```python
from build123d import *

# Parameters (mm, degrees)
SKETCH_1_R      = 11.5
SKETCH_1_R_2    = 6.5
EXTRUDE_1_DEPTH = 14
SKETCH_2_R      = 19
SKETCH_2_R_2    = 6.5
EXTRUDE_2_DEPTH = 12
SKETCH_3_R      = 3.3
EXTRUDE_3_DEPTH = 4


with BuildPart() as part:
    # 草图1 → 拉伸1 (new body)
    with BuildSketch(Plane(origin=(0, 0, 0), x_dir=(1, 0, 0), z_dir=(0, 1, 0))):
        with Locations(Location((0, 0, 0), (0, 0, 270))):
            Circle(SKETCH_1_R)
        with Locations(Location((0, 0, 0), (0, 0, 270))):
            Circle(SKETCH_1_R_2, mode=Mode.SUBTRACT)
    extrude(amount=EXTRUDE_1_DEPTH)

    # 草图2 → 拉伸2 (add)
    with BuildSketch(Plane(origin=(0, 14, 0), x_dir=(-1, 0, 0), z_dir=(0, 1, 0))):
        with Locations(Location((0, 0, 0), (0, 0, 90))):
            Circle(SKETCH_2_R)
        with Locations(Location((0, 0, 0), (0, 0, 90))):
            Circle(SKETCH_2_R_2, mode=Mode.SUBTRACT)
    extrude(amount=EXTRUDE_2_DEPTH)

    # 草图3 → 拉伸3 (add)
    with BuildSketch(Plane(origin=(0, 26, 0), x_dir=(-1, 0, 0), z_dir=(0, 1, 0))):
        with Locations(Location((-15, 0, 0), (0, 0, 90))):
            Circle(SKETCH_3_R)
        with Locations(Location((0, -15, 0), (0, 0, 90))):
            Circle(SKETCH_3_R)
        with Locations(Location((0, 15, 0), (0, 0, 90))):
            Circle(SKETCH_3_R)
        with Locations(Location((15, 0, 0), (0, 0, 90))):
            Circle(SKETCH_3_R)
    extrude(amount=EXTRUDE_3_DEPTH)


solid = part.part
```
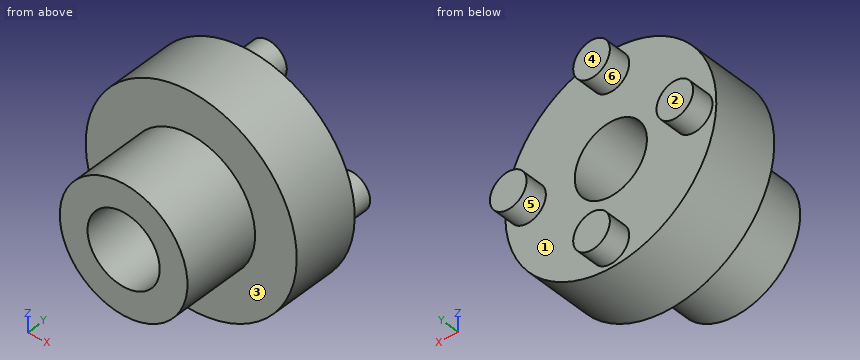
Here's how the part is built. I have some questions about the finished solid (model axes, mm). Face numbers are marked on the shaded views. A direction names the side the tool comes from. Round coordinates to 2 decimals unless told otherwise and drop trailing zeros. Order: outer loops, then holes, each group sorted by start corner. A loop starts at its lowest first (then second) coordinate and runs counter-clockwise, first axis right, second up. Notation, with made-up numbers: (-36, 63) -> (21, 63) arc R25 cw to (21, 101) -> close; hole circle Ø10 at (36, 63). An arc over 180 degrees is marked (long way). Use a Markdown table: item, result. Add a question column.
(1) For the marked faces 1, 2 and 3, which set-ups out of +Z, -Z, +X, -X, +Y, -Y let a thin tool reach every point of the face, with its end or its side?
(2) If we mould it in two halves opening along X, with no side actions, what happens to the marked faces 4, 5 and 6? For each: released by +X, released by -X, zero draft, split by the parting line, or undercut.
(3) For pin 1 Ø1 at (y, z) = (5.5, 6.5) entering from -X; pin 2 Ø3 at (x, z) = (-13, 6.5) entering from +Y; pin 3 Ø12 at (y, z) = (22.5, 11.5) entering from -X, each with a flat end and sliding along its axis, tell me the tip position at first contact or that it passes through.
(4) Suppose I cut it at A-A, the plane z = 0. Please give me the cut outline in (x, y), and give its area (3 significant figures).
(5) Suppose I cut it at B-B, the plane x = 0. Please give me the cut outline in (y, z).
(6) Suppose I cut it at C-C, the plane y = 5.75. Please give me the cut outline in (x, z).
(7) I need wall thicknesses on line 1 along X through (y, z) = (11.5, 0); line 2 along X through (y, z) = (19.5, 0); line 3 along Y through (x, z) = (-15, -5). Which ranges of each line are inside material? Lowest first, please.
(8) Suppose I cut it at D-D, the plane x = -15. Please give me the cut outline in (y, z), and give its area (3 significant figures).
Verdict:
| question | item | result |
|---|---|---|
| 1 | face 1 | +Y |
| 1 | face 2 | +Z, -Z, +X, -X, +Y |
| 1 | face 3 | -Y |
| 2 | face 4 | zero draft |
| 2 | face 5 | undercut |
| 2 | face 6 | split by the parting line |
| 3 | pin 1 | x = -9.81 |
| 3 | pin 2 | y = 26 |
| 3 | pin 3 | x = -18.19 |
| 4 | outline | (-19, 14) -> (-11.5, 14) -> (-11.5, 0) -> (-6.5, 0) -> (-6.5, 26) -> (-11.7, 26) -> (-11.7, 30) -> (-18.3, 30) -> (-18.3, 26) -> (-19, 26) -> close; (6.5, 0) -> (11.5, 0) -> (11.5, 14) -> (19, 14) -> (19, 26) -> (18.3, 26) -> (18.3, 30) -> (11.7, 30) -> (11.7, 26) -> (6.5, 26) -> close |
| 4 | area | 493 mm2 |
| 5 | outline | (0, -11.5) -> (14, -11.5) -> (14, -19) -> (26, -19) -> (26, -18.3) -> (30, -18.3) -> (30, -11.7) -> (26, -11.7) -> (26, -6.5) -> (0, -6.5) -> close; (0, 6.5) -> (26, 6.5) -> (26, 11.7) -> (30, 11.7) -> (30, 18.3) -> (26, 18.3) -> (26, 19) -> (14, 19) -> (14, 11.5) -> (0, 11.5) -> close |
| 6 | outline | circle Ø23 at (0, 0); hole circle Ø13 at (0, 0) |
| 7 | line 1 | -11.5 to -6.5, 6.5 to 11.5 |
| 7 | line 2 | -19 to -6.5, 6.5 to 19 |
| 7 | line 3 | 14 to 26 |
| 8 | outline | (14, -11.66) -> (26, -11.66) -> (26, -3.3) -> (30, -3.3) -> (30, 3.3) -> (26, 3.3) -> (26, 11.66) -> (14, 11.66) -> close |
| 8 | area | 306 mm2 |
